```python
from build123d import *

# Parameters (mm, degrees)
SKETCH1_W           = 40
SKETCH1_H           = 40
BOSS_EXTRUDE1_DEPTH = 10
FILLET1_R           = 20
CUT_EXTRUDE1_DEPTH  = 58.445626465


with BuildPart() as part:
    # Sketch1 → Boss-Extrude1 (new body)
    with BuildSketch(Plane.XY):
        with Locations((20, 20)):
            Rectangle(SKETCH1_W, SKETCH1_H)
    extrude(amount=BOSS_EXTRUDE1_DEPTH)

    # Fillet1
    fillet1_edges = [part.edges().sort_by_distance(p)[0] for p in [
        (0, 40, 5),
    ]]
    fillet(fillet1_edges, radius=FILLET1_R)

    # Sketch2 → Cut-Extrude1 (cut, through all)
    with BuildSketch(Plane(origin=(0, 0, 0), x_dir=(-1, 0, 0), z_dir=(0, 0, -1))):
        with BuildLine():
            Line((-40, 40), (-20, 40))
            ThreePointArc((-20, 40), (-5.857864376, 34.142135624), (0, 20))
            Line((0, 20), (0, 0))
            Line((0, 0), (-7, 0))
            Line((-7, 0), (-7, 20))
            ThreePointArc((-7, 20), (-10.807611845, 29.192388155), (-20, 33))
            Line((-20, 33), (-40, 33))
            Line((-40, 33), (-40, 40))
        make_face()
    extrude(amount=-CUT_EXTRUDE1_DEPTH, mode=Mode.SUBTRACT)


solid = part.part
```
Here's how the part is built. I have some questions about the finished solid (model axes, mm). Give positions to 0.01 mm unless a question says otherwise; leave off trailing zeros. Order: outer loops, then holes, each group sorted by start corner. A loop starts at its lowest first (then second) coordinate and runs counter-clockwise, first axis right, second up. Notation, with made-up numbers: M 10,62.5 L 26,62.5 A25 cw 26,92.5 Z; hole C -36.5,-25.75 d10. An arc over 180 degrees is marked long. Use a Markdown table: item, result. Add a question column.
1. Suppose I cut it at B-B (y = 28). List the corners of the cut face in (x, z) for me.
2. For pin 1 Ø5 at (y, z) = (27, 2) entering from -X, with a flat end and sliding along its axis, tell me the tip position at first contact or that it passes through.
3. I need wall thicknesses on probe 1 along X at (y, z) = (21, 2); probe 2 along Y at (x, z) = (9.5, 9.25); probe 3 along X at (y, z) = (29.5, 5.25). Which ranges of each line are inside material? Lowest first, please. Write a range as from..to.
4. Suppose I cut it at A-A (z = 2). List the corners of the cut face in (x, y) for me, and give its area (3 significant figures).
Results list:
| question | item | result |
|---|---|---|
| 1 | outline | M 9.75,0 L 40,0 L 40,10 L 9.75,10 Z |
| 2 | pin 1 | stops at x = 7.8 |
| 3 | probe 1 | x = 7.04..40 |
| 3 | probe 2 | y = 0..27.66 |
| 3 | probe 3 | x = 11.13..40 |
| 4 | outline | M 7,0 L 40,0 L 40,33 L 20,33 A13 ccw 7,20 Z |
| 4 | area | 1,050 mm² |
